Design review of the part built by this model. Coordinates are the model's own, in mm. Face numbers are marked on the shaded views. A direction names the side the tool comes from. Give positions to 0.01 mm unless a question says otherwise; leave off trailing zeros. Order: outer loops, then holes, each group sorted by start corner. A loop starts at its lowest first (then second) coordinate and runs counter-clockwise, first axis right, second up. Notation, with made-up numbers: (48.25, 69) -> (54.25, 69) arc R28 ccw to (54.25, 107) -> close; hole circle Ø10 at (72, -33). An arc over 180 degrees is marked (long way). Return JSON: item names as keys, results as strings.
```python
from build123d import *

# Parameters (mm, degrees)
SKETCH1_R           = 5.4
BOSS_EXTRUDE1_DEPTH = 124
CUT_EXTRUDE1_START  = -27
SKETCH2_R           = 5.4
SKETCH2_R_2         = 3.6
CUT_EXTRUDE1_DEPTH  = 27
CHAMFER1_SIZE       = 0.54


with BuildPart() as part:
    # Sketch1 → Boss-Extrude1 (new body)
    with BuildSketch(Plane.XY):
        Circle(SKETCH1_R)
    extrude(amount=BOSS_EXTRUDE1_DEPTH)

    # Sketch2 → Cut-Extrude1 (cut)
    with BuildSketch(Plane.XY.offset(124).offset(CUT_EXTRUDE1_START)):
        Circle(SKETCH2_R)
        Circle(SKETCH2_R_2, mode=Mode.SUBTRACT)
    extrude(amount=CUT_EXTRUDE1_DEPTH, mode=Mode.SUBTRACT)

    # Chamfer1
    chamfer1_edges = [part.edges().sort_by_distance(p)[0] for p in [
        (-5.4, 0, 0),
        (-3.6, 0, 124),
    ]]
    chamfer(chamfer1_edges, length=CHAMFER1_SIZE)


solid = part.part
```
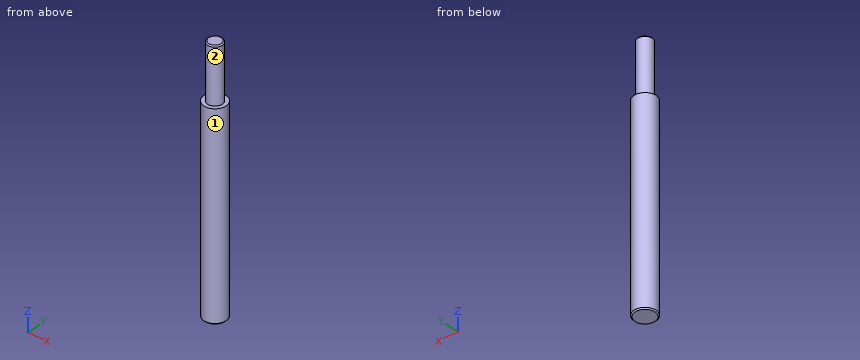
Item 1: Add section C-C (z = 42.5). Give the boundary of the cut face in (x, y).
Result set:
{"outline": "circle Ø10.8 at (0, 0)"}
Item 2: For pin 1 (1.5 mm diameter, centred on y = 2.5, z = 91, fed in from -X); pin 2 (5 mm diameter, centred on y = 3.5, z = 15.5, fed in from -X); pin 3 (3 mm diameter, centred on x = -4, z = 92.5, fed in from -Y), all flat-tipped, find the tip position at first contact; note any pin that passes through.
Result set:
{"pin 1": "stops at x = -5.11", "pin 2": "stops at x = -5.31", "pin 3": "stops at y = -4.79"}
Item 3: Wall thickness on L1, parallel to Z at x = -1.5, y = 3.5; L2, parallel to Y at x = 0.25, z = 8; L3, parallel to Y at x = -3.5, z = 49: over which ranges is each line inside the solid? List them lowest first. Write a range as [from, to].
Result set:
{"L1": "z = [0, 97]", "L2": "y = [-5.39, 5.39]", "L3": "y = [-4.11, 4.11]"}
Item 4: Add section A-A (y = 0). Give the boundary of the cut face in (x, z), plus the area to 3 significant figures.
Result set:
{"outline": "(-5.4, 0.54) -> (-4.86, 0) -> (4.86, 0) -> (5.4, 0.54) -> (5.4, 97) -> (3.6, 97) -> (3.6, 123.46) -> (3.06, 124) -> (-3.06, 124) -> (-3.6, 123.46) -> (-3.6, 97) -> (-5.4, 97) -> close", "area": "1,240 mm^2"}
Item 5: Machinability: for the marked faces 1 and 2, which of the approach directions +Z, -Z, +X, -X, +Y, -Y give a long, thin tool a straight path to every point of the face, cutting with its end or side? Answer none if there is none.
Result set:
{"face 1": "+Z, -Z", "face 2": "+Z"}
